Verification items for the finished model (mm, model axes). A direction names the side the tool comes from. Give positions to 0.01 mm unless a question says otherwise; leave off trailing zeros. Loops run counter-clockwise (first coordinate to the right, second up) from the corner with the lowest first, then second, coordinate; pieces in that order, holes last. Notation, with made-up numbers: M 82.5,43.5 L 95.5,43.5 A32 cw 95.5,75.5 Z; hole C 60.25,35 d10. An arc over 180 degrees is marked long. Use a Markdown table: item, result.
from build123d import *

# Parameters (mm, degrees)
SKETCH1_W           = 268.5
SKETCH1_H           = 155
BOSS_EXTRUDE1_DEPTH = 18
SKETCH2_R           = 5
CUT_EXTRUDE1_DEPTH  = 18
SKETCH3_W           = 100
SKETCH3_H           = 155
CUT_EXTRUDE2_DEPTH  = 10


with BuildPart() as part:
    # Sketch1 → Boss-Extrude1 (new body)
    with BuildSketch(Plane(origin=(0, 0, 0), x_dir=(1, 0, 0), z_dir=(0, 1, 0))):
        Rectangle(SKETCH1_W, SKETCH1_H)
    extrude(amount=BOSS_EXTRUDE1_DEPTH)

    # Sketch2 → Cut-Extrude1 (cut)
    with BuildSketch(Plane(origin=(0, 18, 0), x_dir=(1, 0, 0), z_dir=(0, 1, 0))):
        with Locations(Location((-119.25, 62.5, 0), (0, 0, 270))):
            Circle(SKETCH2_R)
        with Locations(Location((-19.25, 62.5, 0), (0, 0, 270))):
            Circle(SKETCH2_R)
        with Locations(Location((-19.25, -62.5, 0), (0, 0, 90))):
            Circle(SKETCH2_R)
        with Locations(Location((-119.25, -62.5, 0), (0, 0, 90))):
            Circle(SKETCH2_R)
    extrude(amount=-CUT_EXTRUDE1_DEPTH, mode=Mode.SUBTRACT)

    # Sketch3 → Cut-Extrude2 (cut)
    with BuildSketch(Plane(origin=(0, 18, 0), x_dir=(1, 0, 0), z_dir=(0, 1, 0))):
        with Locations((84.25, 0)):
            Rectangle(SKETCH3_W, SKETCH3_H)
    extrude(amount=-CUT_EXTRUDE2_DEPTH, mode=Mode.SUBTRACT)


solid = part.part
(1) Set-up check for faces 5 (the flat face through (34.25, 13, 1)), 6 (the flat face through (-32, 9, 77.5)): record each of +Z, -Z, +X, -X, +Y, -Y from which the full face is reachable in a straight line by a thin tool's end or side.
Results below:
| item | result |
|---|---|
| face 5 | +Z, -Z, +X, +Y |
| face 6 | +Z, +X, -X, +Y, -Y |
(2) Material ranges on line 1 (X direction, y = 9, z = 62.5); line 2 (X direction, y = 14.25, z = 17.5); line 3 (Y direction, x = 71, z = 22), recorded low to high.
Results below:
| item | result |
|---|---|
| line 1 | -134.25 to -124.25, -114.25 to -24.25, -14.25 to 34.25 |
| line 2 | -134.25 to 34.25 |
| line 3 | 0 to 8 |
(3) Cross-section at C-C on x = -19.25. Record the cut outline in (y, z), then the cut area to 3 significant figures.
Results below:
| item | result |
|---|---|
| outline | M 0,-77.5 L 18,-77.5 L 18,-67.5 L 0,-67.5 Z; M 0,-57.5 L 18,-57.5 L 18,57.5 L 0,57.5 Z; M 0,67.5 L 18,67.5 L 18,77.5 L 0,77.5 Z |
| area | 2,430 mm^2 |
(4) Cross-section at B-B on y = 10.5. Record the cut outline in (x, z).
Results below:
| item | result |
|---|---|
| outline | M -134.25,-77.5 L 34.25,-77.5 L 34.25,77.5 L -134.25,77.5 Z; hole C -119.25,-62.5 d10; hole C -119.25,62.5 d10; hole C -19.25,-62.5 d10; hole C -19.25,62.5 d10 |
(5) Cross-section at D-D on z = 21. Record the cut outline in (x, y), then the cut area to 3 significant figures.
Results below:
| item | result |
|---|---|
| outline | M -134.25,0 L 134.25,0 L 134.25,8 L 34.25,8 L 34.25,18 L -134.25,18 Z |
| area | 3,830 mm^2 |
(6) Gauge pin test, flat ends, axial feed: P1, Ø4, axis at x = 96, z = 56, coming from the +Y side; P2, Ø4, axis at y = 13.5, z = -10.5, coming from the +X side; P3, Ø9, axis at x = -119.25, z = -62.5, coming from the -Y side. Record the tip position at first contact, or that the pin passes through.
Results below:
| item | result |
|---|---|
| P1 | y = 8 |
| P2 | x = 34.25 |
| P3 | through |
(7) Cross-section at A-A on z = 62.5. Record the cut outline in (x, y).
Results below:
| item | result |
|---|---|
| outline | M -134.25,0 L -124.25,0 L -124.25,18 L -134.25,18 Z; M -114.25,0 L -24.25,0 L -24.25,18 L -114.25,18 Z; M -14.25,0 L 134.25,0 L 134.25,8 L 34.25,8 L 34.25,18 L -14.25,18 Z |
(8) Draft check along Z on faces 1 (the cylindrical face through (-22.29, 9.13, -66.47)), 2 (the flat face through (-32, 9, -77.5)), 3 (the flat face through (-134.25, 9, 1)), 4 (the cylindrical face through (-16.21, 9.13, 66.47)). Enter one of: +Z half, -Z half, draft (parallel to the pull), parting line (faces both ways), or undercut.
Results below:
| item | result |
|---|---|
| face 1 | undercut |
| face 2 | -Z half |
| face 3 | draft |
| face 4 | undercut |
